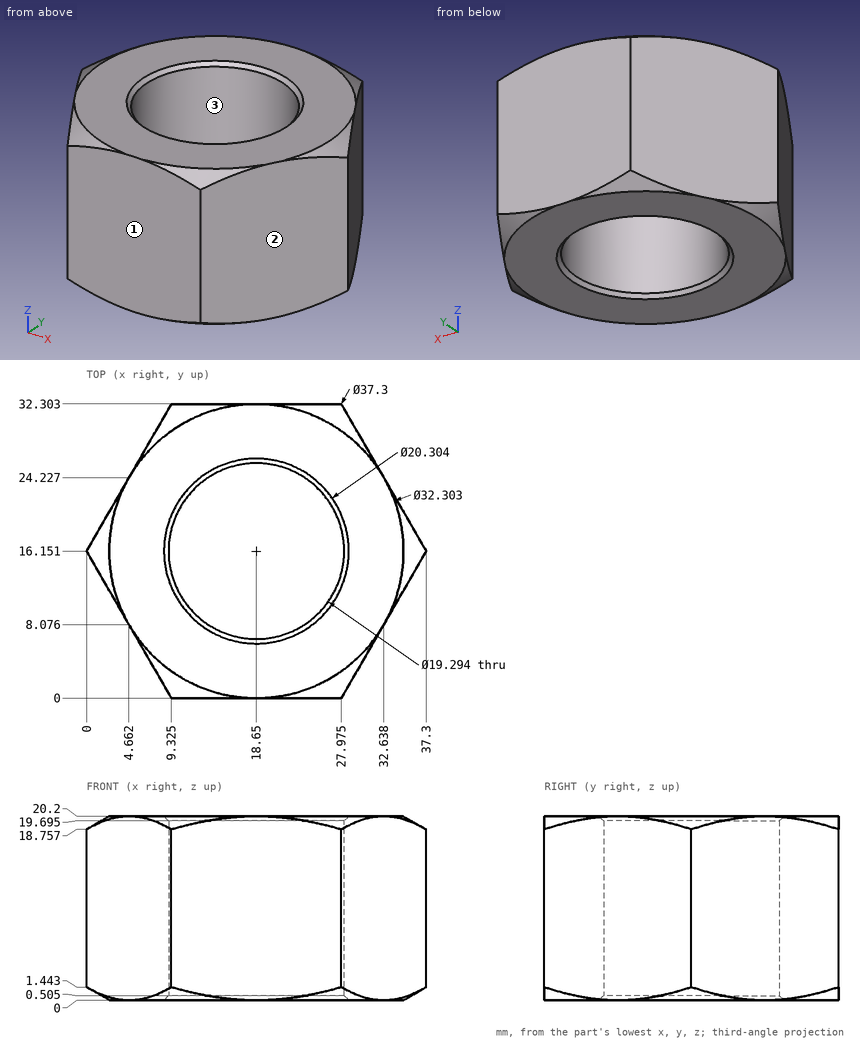
Print and shaded views of the part. All mm, measured from the part's lowest x, y and z. Coordinates: 2 decimals unless noted, no trailing zeros.
(1) Drill centre lines: probe 1 along X at (y, z) = (15.5, 7) (1 decimal); probe 2 along X at (y, z) = (14, 6) (1 decimal); probe 3 along Y at (x, z) = (13.5, 6.5) (1 decimal). Where is each one in solid material? Low to high.
(2) Two-plate mould, pull along X, no slides. Class the marked faces 1, 2 and 3: +X half, -X half, draft (parallel to the pull), parting line (faces both ways), or undercut.
(3) Flat gauge pins, fed straight in: pin 1 (3 mm diameter, centred on y = 13, z = 6.5, fed in from -X); pin 2 (1 mm diameter, centred on x = 33, z = 16.5, fed in from +Y) (1 decimal); pin 3 (1.5 mm diameter, centred on y = 12, z = 9.5, fed in from -X) (1 decimal). Where does each tip first touch, or does it go through?
Geometry says:
1. probe 1: x = 0.4 to 9, 28.3 to 36.9
1. probe 2: x = 1.2 to 9.2, 28.1 to 36.1
1. probe 3: y = 0 to 8, 24.3 to 32.3
2. face 1: draft
2. face 2: +X half
2. face 3: undercut
3. pin 1: stops at x = 0.95
3. pin 2: stops at y = 24.5
3. pin 3: stops at x = 2
